Geometry: final body of the model. Coordinates: model frame, mm. A direction names the side the tool comes from. Give positions to 0.01 mm unless a question says otherwise; leave off trailing zeros. Write each loop counter-clockwise with the first axis right and the second up, starting at its lowest first coordinate (ties: lowest second). Pieces come first, ordered by that corner, then holes. Notation, with made-up numbers: M 59.25,-11.5 L 109.25,-11.5 A22 cw 109.25,14.5 Z; hole C 17,89.5 d8. An arc over 180 degrees is marked long. Use a Markdown table: item, result. Add a question column.
1) Pin query (flat end, axial travel): pin 1 (1.5 mm diameter, centred on y = 3.5, z = 31, fed in from -X); pin 2 (7 mm diameter, centred on x = -37.5, z = 13, fed in from -Y); pin 3 (1.5 mm diameter, centred on x = -26.5, y = 3, fed in from +Z). Return the tip coordinate at first contact, or that it passes through.
2) Set-up query: faces 1 (the flat face through (-33, 3, 23.5)), 2 (the cylindrical face through (35.42, 2.47, -28.01)). Return all of +Z, -Z, +X, -X, +Y, -Y with unobstructed straight access to the full face (end or side cutting, diameter ignored); none if empty.
3) Section A-A on z = -32. Return the cut outline in (x, y), then the cut area to 3 significant figures.
4) Section D-D on x = -31. Return the cut outline in (y, z), then the cut area to 3 significant figures.
5) Draft query along Z for faces 3 (the flat face through (-15, 3, 33)), 4 (the cylindrical face through (-41.792, 2.465, 11.648)), 5 (the cylindrical face through (-48.57, 2.46, 22)). Return one class per face: +Z half, -Z half, draft (parallel to the pull), parting line (faces both ways), or undercut.
6) Line query: line 1 (X direction, y = 3.45, z = -32); line 2 (Z direction, x = -37.5, y = 1.5); line 3 (Z direction, x = 37.5, y = 1.7). Output: solid intervals per line, ascending.
7) Section B-B on x = 37.5. Return the cut outline in (y, z).
8) Section C-C on y = 3.1. Return the cut outline in (x, z), then the cut area to 3 significant figures.
```python
from build123d import *

# Parameters (mm, degrees)
SKETCH2_W            = 100
SKETCH2_H            = 85
BOSS_EXTRUDE1_DEPTH  = 5
M8_CLEARANCE_HOLE1_D = 9
FILLET1_R            = 5
SKETCH7_W            = 35
SKETCH7_H            = 19
CUT_EXTRUDE1_DEPTH   = 5
FILLET2_R            = 5


with BuildPart() as part:
    # Sketch2 → Boss-Extrude1 (new body)
    with BuildSketch(Plane(origin=(0, 0, 0), x_dir=(1, 0, 0), z_dir=(0, 1, 0))):
        Rectangle(SKETCH2_W, SKETCH2_H)
    extrude(amount=BOSS_EXTRUDE1_DEPTH)

    # M8 Clearance Hole1 (through all)
    with Locations(Plane(origin=(0, 5, 0), x_dir=(1, 0, 0), z_dir=(0, 1, 0))):
        with Locations((-37.5, 32), (37.5, 32), (37.5, -13), (-37.5, -13)):
            Hole(M8_CLEARANCE_HOLE1_D / 2)

    # Fillet1
    fillet1_edges = [part.edges().sort_by_distance(p)[0] for p in [
        (50, 2.5, 42.5),
        (-50, 2.5, -42.5),
        (50, 2.5, -42.5),
    ]]
    fillet(fillet1_edges, radius=FILLET1_R)

    # Sketch7 → Cut-Extrude1 (cut)
    with BuildSketch(Plane(origin=(0, 5, 0), x_dir=(1, 0, 0), z_dir=(0, 1, 0))):
        with Locations((-32.5, -33)):
            Rectangle(SKETCH7_W, SKETCH7_H)
    extrude(amount=-CUT_EXTRUDE1_DEPTH, mode=Mode.SUBTRACT)

    # Fillet2
    fillet2_edges = [part.edges().sort_by_distance(p)[0] for p in [
        (-50, 2.5, 23.5),
        (-15, 2.5, 23.5),
        (-15, 2.5, 42.5),
    ]]
    fillet(fillet2_edges, radius=FILLET2_R)


solid = part.part
```
Found:
| question | item | result |
|---|---|---|
| 1 | pin 1 | x = -15 |
| 1 | pin 2 | through |
| 1 | pin 3 | z = 23.5 |
| 2 | face 1 | +Z, -X, +Y, -Y |
| 2 | face 2 | +Y, -Y |
| 3 | outline | M -50,0 L -42,0 L -42,5 L -50,5 Z; M -33,0 L 33,0 L 33,5 L -33,5 Z; M 42,0 L 50,0 L 50,5 L 42,5 Z |
| 3 | area | 410 mm² |
| 4 | outline | M 0,-42.5 L 5,-42.5 L 5,23.5 L 0,23.5 Z |
| 4 | area | 330 mm² |
| 5 | face 3 | draft |
| 5 | face 4 | undercut |
| 5 | face 5 | +Z half |
| 6 | line 1 | -50 to -42, -33 to 33, 42 to 50 |
| 6 | line 2 | -42.5 to -36.5, -27.5 to 8.5, 17.5 to 23.5 |
| 6 | line 3 | -42.5 to -36.5, -27.5 to 8.5, 17.5 to 42.5 |
| 7 | outline | M 0,-42.5 L 5,-42.5 L 5,-36.5 L 0,-36.5 Z; M 0,-27.5 L 5,-27.5 L 5,8.5 L 0,8.5 Z; M 0,17.5 L 5,17.5 L 5,42.5 L 0,42.5 Z |
| 8 | outline | M -50,-37.5 A5 ccw -45,-42.5 L 45,-42.5 A5 ccw 50,-37.5 L 50,37.5 A5 ccw 45,42.5 L -10,42.5 A5 ccw -15,37.5 L -15,28.5 A5 cw -20,23.5 L -45,23.5 A5 ccw -50,18.5 Z; hole C -37.5,-32 d9; hole C -37.5,13 d9; hole C 37.5,-32 d9; hole C 37.5,13 d9 |
| 8 | area | 7,560 mm² |
